from build123d import *

# Parameters (mm, degrees)
BASE_CYLINDER_SKETCH_R         = 30
BASE_CYLINDER_SKETCH_R_2       = 15
BASE_CYLINDER_60_DEPTH         = 20
SUPPORT_ARM_DEPTH              = 30
HUB_BOSS_A_SKETCH_R            = 30
HUB_BOSS_A_DEPTH               = 10
HUB_BOSS_B_SKETCH_R            = 30
HUB_BOSS_B_DEPTH               = 10
ARM_PAD_SKETCH_R               = 30
ARM_PAD_SKETCH_R_2             = 15
ARM_PAD_DEPTH                  = 10
ARM_BOSS_SKETCH_R              = 30
ARM_BOSS_DEPTH                 = 10
SUPPORT_RIB_12MM_DEPTH         = 6
ARM_POCKET_CUT_DEPTH           = 40
TAPERED_BOSS_SKETCH_R          = 30
TAPERED_BOSS_14DEG_DRAFT_DEPTH = 40
TAPERED_BOSS_14DEG_DRAFT_TAPER = 14
BOSS_HOLE_SKETCH_R             = 10
BOSS_HOLE_20_DEPTH             = 177.046816624
CYLINDER_BORE_SKETCH_R         = 15.308926848
CYLINDER_BORE_DEPTH            = 163.449944447


with BuildPart() as part:
    # Base Cylinder Sketch → Base Cylinder Ø60 (new, symmetric)
    with BuildSketch(Plane.XY):
        Circle(BASE_CYLINDER_SKETCH_R)
        Circle(BASE_CYLINDER_SKETCH_R_2, mode=Mode.SUBTRACT)
    extrude(amount=BASE_CYLINDER_60_DEPTH, both=True)

    # Support Arm Sketch → Support Arm (add, symmetric)
    with BuildSketch(Plane.XY):
        with BuildLine():
            Line((-28.708286934, 56.708286934), (-28.708286934, 8.708286934))
            ThreePointArc((-28.708286934, 8.708286934), (-21.213203436, 21.213203436), (-8.708286934, 28.708286934))
            Line((-8.708286934, 28.708286934), (-8.708286934, 76.708286934))
            Line((-8.708286934, 76.708286934), (-88.708286934, 76.708286934))
            Line((-88.708286934, 76.708286934), (-88.708286934, 56.708286934))
            Line((-88.708286934, 56.708286934), (-28.708286934, 56.708286934))
        make_face()
    extrude(amount=SUPPORT_ARM_DEPTH, both=True)

    # Hub Boss A Sketch → Hub Boss A (add, symmetric)
    with BuildSketch(Plane.XY.offset(20)):
        Circle(HUB_BOSS_A_SKETCH_R)
    extrude(amount=HUB_BOSS_A_DEPTH, both=True)

    # Hub Boss B Sketch → Hub Boss B (add, symmetric)
    with BuildSketch(Plane(origin=(0, 0, -20), x_dir=(-1, 0, 0), z_dir=(0, 0, -1))):
        Circle(HUB_BOSS_B_SKETCH_R)
    extrude(amount=HUB_BOSS_B_DEPTH, both=True)

    # Arm Pad Sketch → Arm Pad (add, symmetric)
    with BuildSketch(Plane.XY.offset(30)):
        with Locations(Location((0, 0, 0), (0, 0, 163.125505702))):
            Circle(ARM_PAD_SKETCH_R)
        Circle(ARM_PAD_SKETCH_R_2, mode=Mode.SUBTRACT)
    extrude(amount=ARM_PAD_DEPTH, both=True)

    # Arm Boss Sketch → Arm Boss (add, symmetric)
    with BuildSketch(Plane(origin=(0, 0, -30), x_dir=(-1, 0, 0), z_dir=(0, 0, -1))):
        Circle(ARM_BOSS_SKETCH_R)
    extrude(amount=ARM_BOSS_DEPTH, both=True)

    # Rib Profile Sketch → Support Rib 12mm (add, symmetric)
    with BuildSketch(Plane.XY):
        with BuildLine():
            Line((-8.708286934, 76.708286934), (-8.708286934, 28.708286934))
            ThreePointArc((-8.708286934, 28.708286934), (10.568877445, 28.076659872), (25.477478309, 15.839763225))
            Line((25.477478309, 15.839763225), (-8.708286934, 76.708286934))
        make_face()
    extrude(amount=SUPPORT_RIB_12MM_DEPTH, both=True)

    # Arm Pocket Sketch → Arm Pocket Cut (cut)
    with BuildSketch(Plane(origin=(0, 76.708286934, 0), x_dir=(1, 0, 0), z_dir=(0, 1, 0))):
        with BuildLine():
            Line((-88.708286934, -30), (-58.708286934, -30))
            ThreePointArc((-58.708286934, -30), (-79.921490343, -21.213203462), (-88.708286934, -7.5e-08))
            Line((-88.708286934, -7.5e-08), (-88.708286934, -30))
        make_face()
        with BuildLine():
            Line((-88.708286934, 30), (-88.708286934, -7.5e-08))
            ThreePointArc((-88.708286934, -7.5e-08), (-79.921490396, 21.213203409), (-58.708286934, 30))
            Line((-58.708286934, 30), (-88.708286934, 30))
        make_face()
    extrude(amount=-ARM_POCKET_CUT_DEPTH, mode=Mode.SUBTRACT)

    # Tapered Boss Sketch → Tapered Boss 14deg Draft (add)
    with BuildSketch(Plane(origin=(0, 76.708286934, 0), x_dir=(1, 0, 0), z_dir=(0, 1, 0))):
        with Locations((-58.708286934, 0)):
            Circle(TAPERED_BOSS_SKETCH_R)
    extrude(amount=TAPERED_BOSS_14DEG_DRAFT_DEPTH, taper=TAPERED_BOSS_14DEG_DRAFT_TAPER)

    # Boss Hole Sketch → Boss Hole Ø20 (cut, through all)
    with BuildSketch(Plane(origin=(0, 116.708286934, 0), x_dir=(1, 0, 0), z_dir=(0, 1, 0))):
        with Locations(Location((-59.262949737, 0, 0), (0, 0, 180))):
            Circle(BOSS_HOLE_SKETCH_R)
    extrude(amount=-BOSS_HOLE_20_DEPTH, mode=Mode.SUBTRACT)

    # Cylinder Bore Sketch → Cylinder Bore (cut, through all)
    with BuildSketch(Plane.XY.offset(30)):
        Circle(CYLINDER_BORE_SKETCH_R)
    extrude(amount=-CYLINDER_BORE_DEPTH, mode=Mode.SUBTRACT)


solid = part.part
Work out the finished part from the listing and answer in its coordinate system (mm). A direction names the side the tool comes from. Give positions to 0.01 mm unless a question says otherwise; leave off trailing zeros. Write each loop counter-clockwise with the first axis right and the second up, starting at its lowest first coordinate (ties: lowest second). Pieces come first, ordered by that corner, then holes.
Q1. The part is cut by section C-C on y = -7.5. Give the vertices of the cut face in (x, z).
Answer:
outline: (-29.05, -40) - (-13.35, -40) - (-13.35, 30) - (-12.99, 30) - (-12.99, 40) - (-29.05, 40) - close; (12.99, 30) - (13.35, 30) - (13.35, -40) - (29.05, -40) - (29.05, 40) - (12.99, 40) - close
Q2. The part is cut by section A-A on x = -1. Give the vertices of the cut face in (y, z), and give its area (3 significant figures).
Answer:
outline: (-29.98, -40) - (-15.28, -40) - (-15.28, 30) - (-14.97, 30) - (-14.97, 40) - (-29.98, 40) - close; (14.97, 30) - (15.28, 30) - (15.28, -40) - (29.98, -40) - (29.98, -6) - (62.98, -6) - (62.98, 6) - (29.98, 6) - (29.98, 40) - (14.97, 40) - close
area: 2,760 mm2
Q3. The part is cut by section D-D on y = 63. Give the vertices of the cut face in (x, z), and give its area (3 significant figures).
Answer:
outline: (-58.71, -30) - (-8.71, -30) - (-8.71, -6) - (-1.01, -6) - (-1.01, 6) - (-8.71, 6) - (-8.71, 30) - (-58.71, 30) arc R30 ccw to start; hole circle Ø20 at (-59.26, 0)
area: 4,190 mm2
Q4. Given pin 1 (10.5 mm diameter, centred on x = 16.5, y = 42, fed in from -Z); pin 2 (6 mm diameter, centred on x = -16, z = 27.5, fed in from +Y); pin 3 (5 mm diameter, centred on y = 26, z = 28.5, fed in from -X), each flat-ended and moving along its own axis, determine where each tip first touches the part or whether it passes through.
Answer:
pin 1: stops at z = -6
pin 2: stops at y = 76.71
pin 3: stops at x = -28.71
Q5. A tool of negligible diameter and unlimited length cuts with its end or side. For faces 1 (the face through (-28.5, 50.7, -30)), 2 (the face through (-28.708, 33, 0)), 3 (the face through (10.1, -11.3, 30)), from which of +Z, -Z, +X, -X, +Y, -Y can it reach the whole face along a straight path? Write none if from no direction.
Answer:
face 1: -Z, -X, +Y
face 2: +Z, -Z, -X
face 3: -Z
Q6. Straight lines are drawn through the part: L1, parallel to Y at x = 0, z = 36.5; L2, parallel to Y at x = 0, z = 15. For each, find the intervals that lie inside material, in ascending order.
Answer:
L1: y = -30 to -15, 15 to 30
L2: y = -30 to -15.31, 15.31 to 30
Q7. The part is cut by section B-B on z = -33. Give the vertices of the cut face in (x, y), and give its area (3 significant figures).
Answer:
outline: circle Ø60 at (0, 0); hole circle Ø30.62 at (0, 0)
area: 2,090 mm2
Q8. For a pull along X with two mould halves and no side action, classify faces 4 (the face through (-22, 76.708, 0)), 5 (the face through (8.624, 45.848, 0.084)), 6 (the face through (-1.99, 15.18, -4.51)) as released by +X, released by -X, zero draft, split by the parting line, or undercut.
Answer:
face 4: zero draft
face 5: released by +X
face 6: undercut
